from build123d import *

# Parameters (mm, degrees)
EXTRUDE_1_DEPTH        = 10
HOLE_WIZARD_M5_2_D     = 4.2
HOLE_WIZARD_M5_2_DEPTH = 13
HOLE_WIZARD_M5_2_TIP   = 1.2618073
HOLE_WIZARD_M5_1_D     = 4.2
HOLE_WIZARD_M5_1_DEPTH = 13
HOLE_WIZARD_M5_1_TIP   = 1.2618073
CHAMFER_1_SIZE         = 2


with BuildPart() as part:
    # 草图1 → 凸台-拉伸1 (new body)
    with BuildSketch(Plane.XY):
        Polygon((-64.634074155, -10.796814071), (-39.634074155, -10.796814071), (-39.634074155, -25.796814071), (-55.634074155, -46.796814071), (-64.634074155, -46.796814071), align=None)
    extrude(amount=EXTRUDE_1_DEPTH)

    # M5 螺纹孔2
    with Locations(Plane(origin=(0, -10.796814071, 0), x_dir=(1, 0, 0), z_dir=(0, 1, 0))):
        with Locations((-47.634074155, -5)):
            Hole(HOLE_WIZARD_M5_2_D / 2, depth=HOLE_WIZARD_M5_2_DEPTH)
            with Locations((0, 0, -(HOLE_WIZARD_M5_2_DEPTH + HOLE_WIZARD_M5_2_TIP / 2))):  # 118° drill point
                Cone(0, HOLE_WIZARD_M5_2_D / 2, HOLE_WIZARD_M5_2_TIP, mode=Mode.SUBTRACT)

    # M5 螺纹孔1
    with Locations(Plane.ZY.offset(64.634074155)):
        with Locations((5, -18.796814071), (5, -38.796814071)):
            Hole(HOLE_WIZARD_M5_1_D / 2, depth=HOLE_WIZARD_M5_1_DEPTH)
            with Locations((0, 0, -(HOLE_WIZARD_M5_1_DEPTH + HOLE_WIZARD_M5_1_TIP / 2))):  # 118° drill point
                Cone(0, HOLE_WIZARD_M5_1_D / 2, HOLE_WIZARD_M5_1_TIP, mode=Mode.SUBTRACT)

    # 倒角1
    chamfer_1_edges = [part.edges().sort_by_distance(p)[0] for p in [
        (-64.634074155, -10.796814071, 5),
    ]]
    chamfer(chamfer_1_edges, length=CHAMFER_1_SIZE)


solid = part.part
Part model, mm, in its own coordinate system. A direction names the side the tool comes from. Round coordinates to 2 decimals unless told otherwise and drop trailing zeros. Loops run counter-clockwise (first coordinate to the right, second up) from the corner with the lowest first, then second, coordinate; pieces in that order, holes last. Notation, with made-up numbers: (31, -24.75) - (89, -24.75) arc R28 cw to (89, 11.25) - close; hole circle Ø11 at (50, -5.5). An arc over 180 degrees is marked (long way). Answer as a JSON object with one key per item and string values.
Item 1: Pull direction Y, two halves, no side cores. Call faces 4 (the face through (-58.043, -17.026, 3.871)), 5 (the face through (-55, -25, 0)), 6 (the face through (-47.9, -24.84, 4.75)), 7 (the face through (-47.52, -36.15, 4.93)): pulls with the +Y half, pulls with the -Y half, needs draft (parallel to the pull), parting line crosses it, or undercut.
Output:
{"face 4": "undercut", "face 5": "needs draft", "face 6": "pulls with the +Y half", "face 7": "pulls with the -Y half"}
Item 2: Tool access for faces 1 (the face through (-51, -10.797, 5)), 2 (the face through (-58.04, -40.07, 6.67)), 3 (the face through (-48.603, -17.388, 6.863)): list every direction of +Z, -Z, +X, -X, +Y, -Y with a clear straight run to the whole face (end or side of a thin tool).
Output:
{"face 1": "+Z, -Z, +X, -X, +Y", "face 2": "-X", "face 3": "+Y"}
Item 3: Band-saw the part on B-B on x = -56.75. List the corners of the cut face in (y, z).
Output:
{"outline": "(-46.8, 0) - (-10.8, 0) - (-10.8, 10) - (-46.8, 10) - close; hole circle Ø4.2 at (-38.8, 5); hole circle Ø4.2 at (-18.8, 5)"}
Item 4: Wall check: L1, parallel to Y at x = -57.75, z = 5; L2, parallel to Y at x = -55.5, z = 5.75; L3, parallel to X at y = -18, z = 4.5. Give the ranges that are in metal, low to high.
Output:
{"L1": "-46.8 to -40.9, -36.7 to -20.9, -16.7 to -10.8", "L2": "-46.62 to -40.76, -36.84 to -20.76, -16.84 to -10.8", "L3": "-50.94 to -49.67, -45.59 to -39.63"}
Item 5: Band-saw the part on A-A on y = -22. List the corners of the cut face in (x, z).
Output:
{"outline": "(-64.63, 0) - (-39.63, 0) - (-39.63, 10) - (-64.63, 10) - close; hole circle Ø4.2 at (-47.63, 5)"}
Item 6: Pin check, flat tips, straight feed: pin 1 (6 mm diameter, centred on x = -42.5, z = 2, fed in from -Y); pin 2 (8 mm diameter, centred on x = -53.5, y = -41, fed in from -Z); pin 3 (3.5 mm diameter, centred on x = -47.63, z = 5, fed in from +Y); pin 4 (2 mm diameter, centred on x = -43.5, z = 5, fed in from -Y). Stop position of each tip, or through.
Output:
{"pin 1": "y = -33.5", "pin 2": "z = 0", "pin 3": "y = -24", "pin 4": "y = -32.18"}
